The model under review builds one solid part; all positions refer to its coordinate system, in mm. Face numbers are marked on the shaded views. A direction names the side the tool comes from. Round coordinates to 2 decimals unless told otherwise and drop trailing zeros. Write each loop counter-clockwise with the first axis right and the second up, starting at its lowest first coordinate (ties: lowest second). Pieces come first, ordered by that corner, then holes. Notation, with made-up numbers: (10, 11.5) -> (25, 11.5) arc R14 ccw to (25, 26.5) -> close; hole circle Ø8 at (31.25, 31). An arc over 180 degrees is marked (long way). Answer in a Markdown table with one row per item. Add a question column.
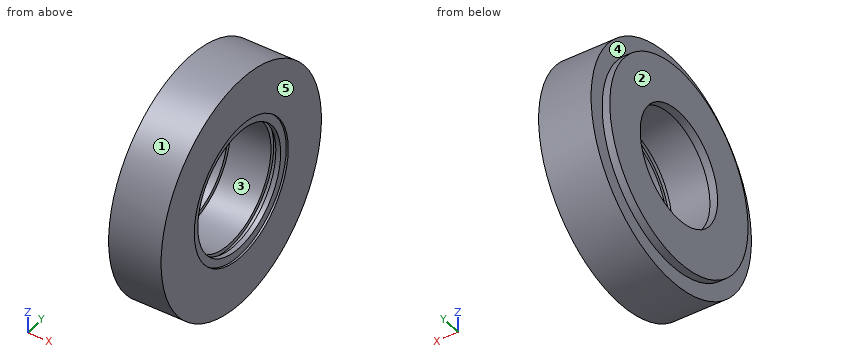
```python
from build123d import *


with BuildPart() as part:
    # 草图2 → 旋转1 (revolve)
    with BuildSketch(Plane.XY, mode=Mode.PRIVATE) as revolve_1_sk:
        Polygon((0, 14), (1.9, 14), (1.9, 15), (12, 15), (12, 16), (13.2, 16), (13.2, 15), (14.4, 15), (14.4, 17), (14.9, 17), (14.9, 29), (1.9, 29), (1.9, 25), (0, 25), align=None)
    revolve(revolve_1_sk.sketch.rotate(Axis((-10.496116508, 0, 0), (1, 0, 0)), 90), axis=Axis((-10.496116508, 0, 0), (1, 0, 0)))


solid = part.part
```
1. Insertion check: pin 1 Ø8 at (x, y) = (12.5, -5) entering from -Z; pin 2 Ø17.5 at (y, z) = (12.5, 6.5) entering from -X; pin 3 Ø2 at (x, z) = (1.5, 21) entering from +Y; pin 4 Ø5 at (x, z) = (1.5, -1) entering from +Y. Each pin has a flat end and moves straight along its axis. Give the tip position at first contact, or say it passes through.
2. Mouldability with a two-part tool opening along Y and no side actions: class the marked faces 1, 2 and 3 as pulls with the +Y half, pulls with the -Y half, needs draft (parallel to the pull), parting line crosses it, or undercut.
3. Add section C-C on x = 8.5. Write out the cut boundary in (y, z), plus the area to 3 significant figures.
4. For L1, parallel to Y at x = 0.55, z = 0; L2, parallel to Y at x = 5.75, z = 0; L3, parallel to Z at x = 4, y = -6, list the stretches that pass through material, from the lowest coordinate up.
5. Add section A-A on y = 0. Write out the cut boundary in (x, z), plus the area to 3 significant figures.
6. Tool access review of the marked faces 4 and 5: name each direction out of +Z, -Z, +X, -X, +Y, -Y from which nothing blocks a thin tool from reaching the whole face with its end or side.
7. Add section D-D on z = 21. Write out the cut boundary in (x, y), plus the area to 3 significant figures.
Filled in:
| question | item | result |
|---|---|---|
| 1 | pin 1 | z = -28.98 |
| 1 | pin 2 | x = 0 |
| 1 | pin 3 | y = 20.92 |
| 1 | pin 4 | y = 29 |
| 2 | face 1 | parting line crosses it |
| 2 | face 2 | needs draft |
| 2 | face 3 | undercut |
| 3 | outline | circle Ø58 at (0, 0); hole circle Ø30 at (0, 0) |
| 3 | area | 1,940 mm² |
| 4 | L1 | -25 to -14, 14 to 25 |
| 4 | L2 | -29 to -15, 15 to 29 |
| 4 | L3 | -28.37 to -13.75, 13.75 to 28.37 |
| 5 | outline | (0, -25) -> (1.9, -25) -> (1.9, -29) -> (14.9, -29) -> (14.9, -17) -> (14.4, -17) -> (14.4, -15) -> (13.2, -15) -> (13.2, -16) -> (12, -16) -> (12, -15) -> (1.9, -15) -> (1.9, -14) -> (0, -14) -> close; (0, 14) -> (1.9, 14) -> (1.9, 15) -> (12, 15) -> (12, 16) -> (13.2, 16) -> (13.2, 15) -> (14.4, 15) -> (14.4, 17) -> (14.9, 17) -> (14.9, 29) -> (1.9, 29) -> (1.9, 25) -> (0, 25) -> close |
| 5 | area | 401 mm² |
| 6 | face 4 | -X |
| 6 | face 5 | +Z, -Z, +X, +Y, -Y |
| 7 | outline | (0, -13.56) -> (1.9, -13.56) -> (1.9, -20) -> (14.9, -20) -> (14.9, 20) -> (1.9, 20) -> (1.9, 13.56) -> (0, 13.56) -> close |
| 7 | area | 572 mm² |
